CAD build for the part. Positions are in the model's coordinates, mm. Face numbers are marked on the shaded views. A direction names the side the tool comes from. Coordinates: 2 decimals unless noted, no trailing zeros. Loops run counter-clockwise (first coordinate to the right, second up) from the corner with the lowest first, then second, coordinate; pieces in that order, holes last. Notation, with made-up numbers: (-33, 82) - (-24, 82) arc R31 ccw to (-24, 120) - close; hole circle Ø8 at (52, -16). An arc over 180 degrees is marked (long way). Put each result on its own line as item: value.
```python
from build123d import *

# Parameters (mm, degrees)
BASE_PLATE_SKETCH_R             = 2.5
POINTED_BASE_PLATE_DEPTH        = 6
BACK_WALL_AND_CLEVIS_LUGS_DEPTH = 25
LUG_BOSS_SKETCH_R               = 8
LUG_BOSS_SKETCH_R_2             = 4
LUG_BOSS_DEPTH                  = 4
PIN_HOLE_REACH                  = 75.058
PIN_HOLE_SKETCH_R               = 4
BASE_MOUNTING_HOLES_REACH       = 67.158
MOUNTING_HOLES_SKETCH_R         = 2.5


with BuildPart() as part:
    # Base Plate Sketch → Pointed Base Plate (new body)
    with BuildSketch(Plane(origin=(0, 0, 0), x_dir=(1, 0, 0), z_dir=(0, 1, 0))):
        with BuildLine():
            Line((-20, 0), (20, 0))
            Line((20, 0), (20, -40))
            Line((20, -40), (5.548667415, -54.451332585))
            ThreePointArc((5.548667415, -54.451332585), (0, -56.749665881), (-5.548667415, -54.451332585))
            Line((-5.548667415, -54.451332585), (-20, -40))
            Line((-20, -40), (-20, 0))
        make_face()
        with Locations(Location((0, -48.902665169, 0), (0, 0, 270))):
            Circle(BASE_PLATE_SKETCH_R, mode=Mode.SUBTRACT)
    extrude(amount=POINTED_BASE_PLATE_DEPTH)

    # Back Wall and Lugs Sketch → Back Wall and Clevis Lugs (add)
    with BuildSketch(Plane(origin=(0, 6, 0), x_dir=(1, 0, 0), z_dir=(0, 1, 0))):
        Polygon((-20, 0), (20, 0), (20, -5), (10, -5), (10, -45), (6, -45), (6, -5), (-6, -5), (-6, -45), (-10, -45), (-10, -5), (-20, -5), align=None)
    extrude(amount=BACK_WALL_AND_CLEVIS_LUGS_DEPTH)

    # Lug Boss Sketch → Lug Boss (add)
    with BuildSketch(Plane(origin=(10, 0, 0), x_dir=(0, 0, -1), z_dir=(1, 0, 0))):
        with Locations(Location((-37, 23, 0), (0, 0, 180))):
            Circle(LUG_BOSS_SKETCH_R)
        with Locations((-37, 23)):
            Circle(LUG_BOSS_SKETCH_R_2, mode=Mode.SUBTRACT)
    lug_boss = extrude(amount=LUG_BOSS_DEPTH)

    # Pin Hole Sketch → Pin Hole (cut, up to next)
    with BuildSketch(Plane(origin=(14, 0, 0), x_dir=(0, 0, -1), z_dir=(1, 0, 0)), mode=Mode.PRIVATE) as pin_hole_sk1:
        with Locations((-37, 23)):
            Circle(PIN_HOLE_SKETCH_R)
    pin_hole_tool1 = extrude(pin_hole_sk1.sketch, amount=-PIN_HOLE_REACH, mode=Mode.PRIVATE) & part.part
    # Pin Hole Sketch → Pin Hole (cut, up to next)
    with BuildSketch(Plane(origin=(14, 0, 0), x_dir=(0, 0, -1), z_dir=(1, 0, 0)), mode=Mode.PRIVATE) as pin_hole_sk2:
        with BuildLine():
            Line((-45, 31), (-45, 23))
            ThreePointArc((-45, 23), (-42.656854249, 28.656854249), (-37, 31))
            Line((-37, 31), (-45, 31))
        make_face()
    pin_hole_tool2 = extrude(pin_hole_sk2.sketch, amount=-PIN_HOLE_REACH, mode=Mode.PRIVATE) & part.part
    pin_hole_1 = pin_hole_tool1.solids().sort_by_distance((14, 23, 37))[0]
    add(pin_hole_1, mode=Mode.SUBTRACT)
    pin_hole_2 = pin_hole_tool2.solids().sort_by_distance((14, 29.213056, 43.213056))[0]
    add(pin_hole_2, mode=Mode.SUBTRACT)
    pin_hole = pin_hole_1 + pin_hole_2  # Pin Hole as one shape, for the pattern or mirror that repeats it

    # Lug Boss and Pin Hole Mirror: Lug Boss, Pin Hole across plane
    add(lug_boss.mirror(Plane(origin=(0, 0, 0), x_dir=(0, 0, 1), z_dir=(1, 0, 0))))
    add(pin_hole.mirror(Plane(origin=(0, 0, 0), x_dir=(0, 0, 1), z_dir=(1, 0, 0))), mode=Mode.SUBTRACT)

    # Mounting Holes Sketch → Base Mounting Holes (cut, up to next)
    with BuildSketch(Plane(origin=(0, 6, 0), x_dir=(1, 0, 0), z_dir=(0, 1, 0)), mode=Mode.PRIVATE) as base_mounting_holes_sk1:
        with Locations(Location((-15, -15, 0), (0, 0, 270))):
            Circle(MOUNTING_HOLES_SKETCH_R)
    base_mounting_holes_tool1 = extrude(base_mounting_holes_sk1.sketch, amount=-BASE_MOUNTING_HOLES_REACH, mode=Mode.PRIVATE) & part.part
    # Mounting Holes Sketch → Base Mounting Holes (cut, up to next)
    with BuildSketch(Plane(origin=(0, 6, 0), x_dir=(1, 0, 0), z_dir=(0, 1, 0)), mode=Mode.PRIVATE) as base_mounting_holes_sk2:
        with Locations(Location((15, -15, 0), (0, 0, 270))):
            Circle(MOUNTING_HOLES_SKETCH_R)
    base_mounting_holes_tool2 = extrude(base_mounting_holes_sk2.sketch, amount=-BASE_MOUNTING_HOLES_REACH, mode=Mode.PRIVATE) & part.part
    add(base_mounting_holes_tool1.solids().sort_by_distance((-15, 6, 15))[0], mode=Mode.SUBTRACT)
    add(base_mounting_holes_tool2.solids().sort_by_distance((15, 6, 15))[0], mode=Mode.SUBTRACT)


solid = part.part
```
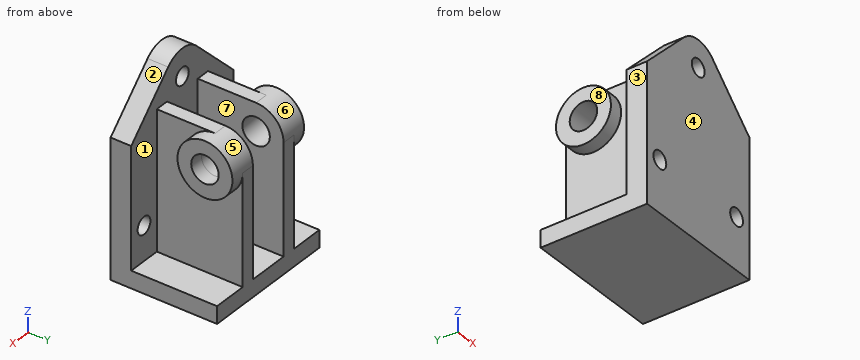
Q1. Slice it at C-C, the plane x = 0. Give the cut face in (y, z).
Determined:
outline: (0, 0) - (31, 0) - (31, 5) - (6, 5) - (6, 46.4) - (0, 46.4) - close; (0, 51.4) - (6, 51.4) - (6, 56.75) - (0, 56.75) - close
Q2. Slice it at D-D, the plane y = 9.5. Give the cut face in (x, z).
Determined:
outline: (-20, 0) - (20, 0) - (20, 5) - (10, 5) - (10, 45) - (6, 45) - (6, 5) - (-6, 5) - (-6, 45) - (-10, 45) - (-10, 5) - (-20, 5) - close
Q3. Mould opens along X. For the marked faces 1, 2, 3 and 4 say: +X half, -X half, draft (parallel to the pull), parting line (faces both ways), or undercut.
Determined:
face 1: undercut
face 2: +X half
face 3: -X half
face 4: draft
Q4. Slice it at A-A, the plane z = 13.5. Give the cut face in (x, y).
Determined:
outline: (-20, 0) - (-17, 0) - (-17, 6) - (-20, 6) - close; (-13, 0) - (13, 0) - (13, 6) - (10, 6) - (10, 31) - (6, 31) - (6, 6) - (-6, 6) - (-6, 31) - (-10, 31) - (-10, 6) - (-13, 6) - close; (17, 0) - (20, 0) - (20, 6) - (17, 6) - close
Q5. Pin check, flat tips, straight feed: pin 1 Ø5 at (y, z) = (21.5, 38) entering from +X; pin 2 Ø12 at (x, y) = (-11.5, 19.5) entering from +Z; pin 3 Ø3 at (x, y) = (-16.5, 21) entering from +Z. Stop position of each tip, or through.
Determined:
pin 1: x = 14
pin 2: z = 45
pin 3: z = 5
Q6. Wall check: L1, parallel to X at y = 2, z = 15; L2, parallel to X at y = 27.5, z = 14; L3, parallel to Z at x = -7, y = 12.5. Give the ranges that are in metal, low to high. Write a range as from..to.
Determined:
L1: -20..-17.5, -12.5..12.5, 17.5..20
L2: -10..-6, 6..10
L3: 0..45
Q7. Tool access for the marked faces 5, 6, 7 and 8: list every direction of +Z, -Z, +X, -X, +Y, -Y with a clear straight run to the whole face (end or side of a thin tool).
Determined:
face 5: +X
face 6: -X
face 7: +Z, +Y
face 8: +Z, -X, +Y
Q8. Slice it at B-B, the plane x = -8. Give the cut face in (y, z).
Determined:
outline: (0, 0) - (31, 0) - (31, 37) arc R8 ccw to (23, 45) - (6, 45) - (6, 52) - (0, 52) - close; hole circle Ø8 at (23, 37)
